The listing builds one solid part. Answer for the finished solid, in the listing's coordinates (mm). Face numbers are marked on the shaded views. A direction names the side the tool comes from. Give positions to 0.01 mm unless a question says otherwise; leave off trailing zeros. Loops run counter-clockwise (first coordinate to the right, second up) from the corner with the lowest first, then second, coordinate; pieces in that order, holes last.
Item 1: Section A-A, the plane x = 0 is taken. Give the vertices of the cut face in (y, z), and give its area (3 significant figures).
Item 2: A tool of negligible diameter and unlimited length cuts with its end or side. For the marked faces 1 and 2, from which of +Z, -Z, +X, -X, +Y, -Y can it reach the whole face along a straight path? Write none if from no direction.
Item 3: Section C-C, the plane y = 39 is taken. Give the vertices of the cut face in (x, z).
Item 4: Consider line 1 along X through (y, z) = (57, 0.25); line 2 along Z through (x, y) = (3.75, 20.5). Determine where each line is inside the solid, lowest interval first.
Item 5: Each of these flat-tipped pins is pushed along its axis until it touches: pin 1 Ø2 at (y, z) = (12, -1) entering from +X; pin 2 Ø1.5 at (x, y) = (0.5, 10.5) entering from -Z; pin 3 Ø4 at (y, z) = (32.5, -3) entering from +X. Where does it stop, or does it pass through?
Item 6: Section B-B, the plane z = 0 is taken. Give the vertices of the cut face in (x, y), and give its area (3 significant figures).
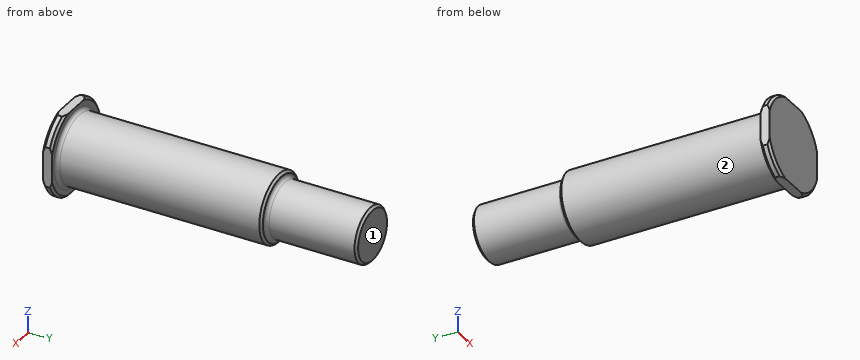
from build123d import *

# Parameters (mm, degrees)
CHAMFER1_SIZE       = 0.5
FILLET1_R           = 0.8
SKETCH2_OUTSIDE_W   = 36.546
SKETCH2_OUTSIDE_H   = 36.546
SKETCH2_OUTSIDE_W_2 = 18
SKETCH2_OUTSIDE_H_2 = 18
CUT_EXTRUDE1_DEPTH  = 10


with BuildPart() as part:
    # Sketch1 → Revolve1 (revolve)
    with BuildSketch(Plane.XY, mode=Mode.PRIVATE) as revolve1_sk:
        Polygon((0, 0), (10, 0), (10, 2), (7.5, 2), (7.5, 47), (6, 47), (6, 67), (0, 67), align=None)
    revolve(revolve1_sk.sketch.rotate(Axis((0, 0, 0), (0, -1, 0)), 90), axis=Axis((0, 0, 0), (0, -1, 0)))

    # Chamfer1
    chamfer1_edges = [part.edges().sort_by_distance(p)[0] for p in [
        (0, 67, -6),
        (0, 47, -7.5),
        (0, 2, -10),
        (0, 0, -10),
    ]]
    chamfer(chamfer1_edges, length=CHAMFER1_SIZE)

    # Fillet1
    fillet1_edges = [part.edges().sort_by_distance(p)[0] for p in [
        (0, 47, -6),
        (0, 2, -7.5),
    ]]
    fillet(fillet1_edges, radius=FILLET1_R)

    # Sketch2 outside → Cut-Extrude1 (cut)
    with BuildSketch(Plane(origin=(0, 0, 0), x_dir=(1, 0, 0), z_dir=(0, 1, 0))):
        Rectangle(SKETCH2_OUTSIDE_W, SKETCH2_OUTSIDE_H)
        Rectangle(SKETCH2_OUTSIDE_W_2, SKETCH2_OUTSIDE_H_2, mode=Mode.SUBTRACT)
    extrude(amount=CUT_EXTRUDE1_DEPTH, mode=Mode.SUBTRACT)


solid = part.part
Worked answers:
1. outline: (0, -9) - (2, -9) - (2, -8.3) arc R0.8 cw to (2.8, -7.5) - (46.5, -7.5) - (47, -7) - (47, -6.8) arc R0.8 cw to (47.8, -6) - (66.5, -6) - (67, -5.5) - (67, 5.5) - (66.5, 6) - (47.8, 6) arc R0.8 cw to (47, 6.8) - (47, 7) - (46.5, 7.5) - (2.8, 7.5) arc R0.8 cw to (2, 8.3) - (2, 9) - (0, 9) - close
1. area: 951 mm2
2. face 1: +Z, -Z, +X, -X, +Y
2. face 2: +Y
3. outline: circle Ø15 at (0, 0)
4. line 1: x = -5.99 to 5.99
4. line 2: z = -6.5 to 6.5
5. pin 1: stops at x = 7.5
5. pin 2: stops at z = -7.5
5. pin 3: stops at x = 7.43
6. outline: (-9, 0) - (9, 0) - (9, 2) - (8.3, 2) arc R0.8 cw to (7.5, 2.8) - (7.5, 46.5) - (7, 47) - (6.8, 47) arc R0.8 cw to (6, 47.8) - (6, 66.5) - (5.5, 67) - (-5.5, 67) - (-6, 66.5) - (-6, 47.8) arc R0.8 cw to (-6.8, 47) - (-7, 47) - (-7.5, 46.5) - (-7.5, 2.8) arc R0.8 cw to (-8.3, 2) - (-9, 2) - close
6. area: 951 mm2
